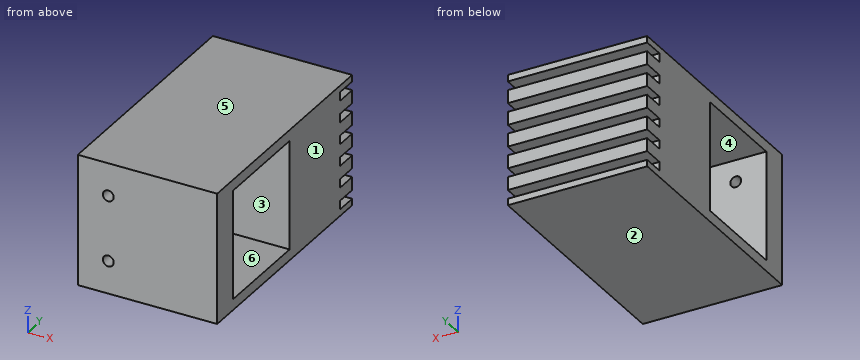
from build123d import *

# Parameters (mm, degrees)
SKETCH_1_W             = 32
SKETCH_1_H             = 30
EXTRUDE_1_DEPTH        = 55
HOLE_WIZARD_M3_1_D     = 2.5
HOLE_WIZARD_M3_1_DEPTH = 7.5
HOLE_WIZARD_M3_1_TIP   = 0.751075774
SKETCH_5_W             = 25
SKETCH_5_H             = 23
CUT_EXTRUDE_2_DEPTH    = 60
SKETCH_6_W             = 2
SKETCH_6_H             = 5
CUT_EXTRUDE_3_DEPTH    = 66.375836515
PATTERN_LINEAR_1_COUNT = 6
PATTERN_LINEAR_1_PITCH = 5


with BuildPart() as part:
    # 草图1 → 凸台-拉伸1 (new body)
    with BuildSketch(Plane(origin=(0, 0, 0), x_dir=(1, 0, 0), z_dir=(0, 1, 0))):
        Rectangle(SKETCH_1_W, SKETCH_1_H)
    extrude(amount=EXTRUDE_1_DEPTH)

    # M3 螺纹孔1
    with Locations(Plane(origin=(0, 0, 0), x_dir=(-1, 0, 0), z_dir=(0, -1, 0))):
        with Locations((9, 7.5), (9, -7.5)):
            Hole(HOLE_WIZARD_M3_1_D / 2, depth=HOLE_WIZARD_M3_1_DEPTH)
            with Locations((0, 0, -(HOLE_WIZARD_M3_1_DEPTH + HOLE_WIZARD_M3_1_TIP / 2))):  # 118° drill point
                Cone(0, HOLE_WIZARD_M3_1_D / 2, HOLE_WIZARD_M3_1_TIP, mode=Mode.SUBTRACT)

    # 草图5 → 切除-拉伸2 (cut)
    with BuildSketch(Plane(origin=(16, 0, 0), x_dir=(0, 0, -1), z_dir=(1, 0, 0))):
        with Locations((0, 18)):
            Rectangle(SKETCH_5_W, SKETCH_5_H)
    extrude(amount=-CUT_EXTRUDE_2_DEPTH, mode=Mode.SUBTRACT)

    # 草图6 → 切除-拉伸3 (cut, through all)
    with BuildSketch(Plane(origin=(16, 0, 0), x_dir=(0, 0, -1), z_dir=(1, 0, 0))):
        with Locations((-12.5, 52.5)):
            Rectangle(SKETCH_6_W, SKETCH_6_H)
    cut_extrude_3 = extrude(amount=-CUT_EXTRUDE_3_DEPTH, mode=Mode.SUBTRACT)

    # 阵列(线性)1: 切除-拉伸3 ×6
    with Locations(*[(0, 0, -i * PATTERN_LINEAR_1_PITCH) for i in range(1, PATTERN_LINEAR_1_COUNT)]):
        add(cut_extrude_3, mode=Mode.SUBTRACT)


solid = part.part
Design review of the part built by this model. Coordinates are the model's own, in mm. Face numbers are marked on the shaded views. A direction names the side the tool comes from. Give positions to 0.01 mm unless a question says otherwise; leave off trailing zeros. Loops run counter-clockwise (first coordinate to the right, second up) from the corner with the lowest first, then second, coordinate; pieces in that order, holes last. Notation, with made-up numbers: M -21,63.5 L 29,63.5 A29 ccw 29,96.5 Z; hole C 1,29 d5. An arc over 180 degrees is marked long. Write item = value, one per line.
Q1. For the marked faces 5 and 6, list the 3-axis set-ups (+Z, -Z, +X, -X, +Y, -Y) from which the entire face can be reached by the end or side of a thin tool; tool diameter is ignored.
Output values:
face_5 = +Z, +X, -X, +Y, -Y
face_6 = +X, -X
Q2. Insertion check: pin 1 (6 mm diameter, centred on x = 3.5, z = 10.5, fed in from -Y); pin 2 (2 mm diameter, centred on x = -9, z = 7.5, fed in from -Y); pin 3 (1 mm diameter, centred on x = -0.5, z = 2.5, fed in from +Y). Each pin has a flat end and moves straight along its axis. Give the tip position at first contact, or say it passes through.
Output values:
pin_1 = 0
pin_2 = 29.5
pin_3 = 50
Q3. We need section C-C (z = -7.5). Give the boundary of the cut face in (x, y).
Output values:
outline = M -16,0 L -10.25,0 L -10.25,6.5 L -16,6.5 Z; M -16,29.5 L 16,29.5 L 16,50 L -16,50 Z; M -7.75,0 L 16,0 L 16,6.5 L -7.75,6.5 Z
Q4. We need section A-A (y = 10.5). Give the boundary of the cut face in (x, z).
Output values:
outline = M -16,-15 L 16,-15 L 16,-12.5 L -16,-12.5 Z; M -16,12.5 L 16,12.5 L 16,15 L -16,15 Z
Q5. To check wall thickness, follow line 1 (Z direction, x = -9, y = 2); line 2 (Y direction, x = 7.5, z = -7.25); line 3 (X direction, y = 2.5, z = -7.5). State the ranges of each line that lie inside material, in increasing order. Write a range as [from, to].
Output values:
line_1 = [-15, -8.75], [-6.25, 6.25], [8.75, 15]
line_2 = [0, 6.5], [29.5, 50]
line_3 = [-16, -10.25], [-7.75, 16]
Q6. Draft analysis for pull direction Z (two halves, no side actions). For the marked faces 1, 2, 3 and 4, state which applies: +Z half, -Z half, draft (parallel to the pull), parting line (faces both ways), or undercut.
Output values:
face_1 = draft
face_2 = -Z half
face_3 = undercut
face_4 = undercut
